```python
from build123d import *

# Parameters (mm, degrees)
EXTRUDE_THIN1_DEPTH = 30
CUT_EXTRUDE1_DEPTH  = 3


with BuildPart() as part:
    # Sketch1 → Extrude-Thin1 (new body)
    with BuildSketch(Plane.XY):
        with BuildLine():
            Line((0, -80), (0, -6))
            ThreePointArc((0, -6), (1.757359313, -1.757359313), (6, 0))
            Line((6, 0), (30, 0))
            Line((30, 0), (30, -3))
            Line((30, -3), (6, -3))
            ThreePointArc((6, -3), (3.878679656, -3.878679656), (3, -6))
            Line((3, -6), (3, -80))
            Line((3, -80), (0, -80))
        make_face()
    extrude(amount=EXTRUDE_THIN1_DEPTH)

    # Sketch2 → Cut-Extrude1 (cut)
    with BuildSketch(Plane.ZY):
        with BuildLine():
            Line((18, -57), (18, -67))
            ThreePointArc((18, -67), (15, -70), (12, -67))
            Line((12, -67), (12, -57))
            ThreePointArc((12, -57), (15, -54), (18, -57))
        make_face()
    extrude(amount=-CUT_EXTRUDE1_DEPTH, mode=Mode.SUBTRACT)


solid = part.part
```
Source: CAD feature listing. Evaluate the final solid. Frame: model axes, mm. A direction names the side the tool comes from. Coordinates: 2 decimals unless noted, no trailing zeros. Loops run counter-clockwise (first coordinate to the right, second up) from the corner with the lowest first, then second, coordinate; pieces in that order, holes last. Notation, with made-up numbers: (46.25, -33.5) -> (56.25, -33.5) arc R17 ccw to (56.25, -27.5) -> close; hole circle Ø8 at (13.25, -17). An arc over 180 degrees is marked (long way). One line per item, written item: value. Start each with the question number.
Q1. Section query D-D, the plane z = 4. Return the cut outline in (x, y).
Q2. Section query C-C, the plane x = 2. Return the cut outline in (y, z), and give its area (3 significant figures).
Q3. Mould query, pull axis Z, two halves, no side actions, for faces 1 (the face through (2, -80, 15)), 2 (the face through (2.8, -30.9, 0)), 3 (the face through (1, -62, 18)). Classes: pulls with the +Z half, pulls with the -Z half, needs draft (parallel to the pull), parting line crosses it, or undercut.
Q4. Contact query for flat-ended pins moving along their axis: P1, Ø4, axis at y = -31.5, z = 12.5, coming from the +X side; P2, Ø12, axis at x = 12.5, z = 19.5, coming from the -Y side. Output: stop coordinate, or through.
Q5. Section query A-A, the plane z = 15. Return the cut outline in (x, y).
Q6. Line query: line 1 along X through (y, z) = (-55, 27); line 2 along Y through (x, z) = (14.75, 21.5); line 3 along Y through (x, z) = (3.75, 3.75). Output: solid intervals per line, ascending.
Q7. Set-up query: faces 4 (the face through (1, -62, 12)), 5 (the face through (18, -3, 15)), 6 (the face through (0, -44, 15)). Return all of +Z, -Z, +X, -X, +Y, -Y with unobstructed straight access to the full face (end or side cutting, diameter ignored); none if empty.
Q8. Section query B-B, the plane y = -64.5. Return the cut outline in (x, z), and give its area (3 significant figures).
Results:
1. outline: (0, -80) -> (3, -80) -> (3, -6) arc R3 cw to (6, -3) -> (30, -3) -> (30, 0) -> (6, 0) arc R6 ccw to (0, -6) -> close
2. outline: (-80, 0) -> (-1.53, 0) -> (-1.53, 30) -> (-80, 30) -> close; hole (-67, 12) -> (-57, 12) arc R3 ccw to (-57, 18) -> (-67, 18) arc R3 ccw to start
2. area: 2,270 mm^2
3. face 1: needs draft
3. face 2: pulls with the -Z half
3. face 3: undercut
4. P1: x = 3
4. P2: y = -3
5. outline: (0, -80) -> (3, -80) -> (3, -70) -> (0, -70) -> close; (0, -54) -> (3, -54) -> (3, -6) arc R3 cw to (6, -3) -> (30, -3) -> (30, 0) -> (6, 0) arc R6 ccw to (0, -6) -> close
6. line 1: 0 to 3
6. line 2: -3 to 0
6. line 3: -4.02 to -0.44
7. face 4: +X, -X
7. face 5: +Z, -Z, +X, -Y
7. face 6: +Z, -Z, -X, +Y, -Y
8. outline: (0, 0) -> (3, 0) -> (3, 12) -> (0, 12) -> close; (0, 18) -> (3, 18) -> (3, 30) -> (0, 30) -> close
8. area: 72.0 mm^2
